```python
from build123d import *

# Parameters (mm, degrees)
CUT_EXTRUDE1_DEPTH = 3
CHAMFER1_SIZE      = 0.5


with BuildPart() as part:
    # Sketch1 → Revolve1 (revolve)
    with BuildSketch(Plane.XY):
        Polygon((0, 0), (0, 6.55), (12, 6.55), (12, 9.5), (17, 9.5), (17, 0), align=None)
    revolve(axis=Axis((17, 0, 0), (-1, 0, 0)))

    # Sketch2 → Cut-Extrude1 (cut)
    with BuildSketch(Plane(origin=(17, 0, 0), x_dir=(0, 0, -1), z_dir=(1, 0, 0))):
        Polygon((0, 4.041451884), (-3.5, 2.020725942), (-3.5, -2.020725942), (0, -4.041451884), (3.5, -2.020725942), (3.5, 2.020725942), align=None)
    extrude(amount=-CUT_EXTRUDE1_DEPTH, mode=Mode.SUBTRACT)

    # Chamfer1
    chamfer1_edges = [part.edges().sort_by_distance(p)[0] for p in [
        (17, -9.5, 0),
        (12, -9.5, 0),
        (0, -6.55, 0),
    ]]
    chamfer(chamfer1_edges, length=CHAMFER1_SIZE)


solid = part.part
```
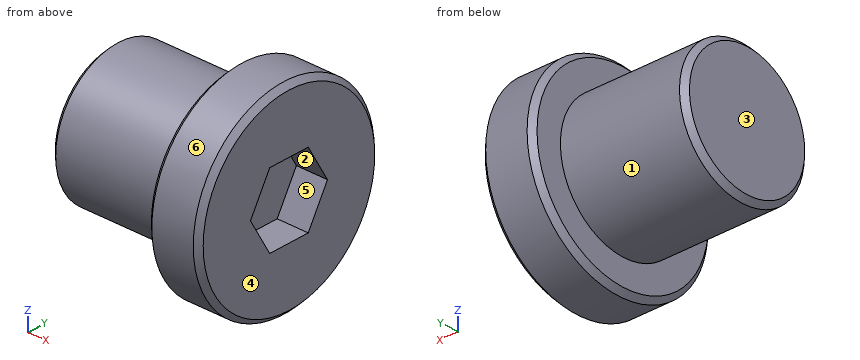
The listing builds one solid part. Answer for the finished solid, in the listing's coordinates (mm). Face numbers are marked on the shaded views. A direction names the side the tool comes from. Round coordinates to 2 decimals unless told otherwise and drop trailing zeros. Order: outer loops, then holes, each group sorted by start corner. A loop starts at its lowest first (then second) coordinate and runs counter-clockwise, first axis right, second up. Notation, with made-up numbers: (89.25, 29) -> (113.25, 29) arc R28 cw to (113.25, 59) -> close; hole circle Ø3 at (49, 73). An arc over 180 degrees is marked (long way). Answer as CSV lines item,"result".
Q1. Consider line 1 (X direction, y = -3.75, z = -4.75); line 2 (X direction, y = 8.5, z = 1.25); line 3 (Y direction, x = 9, z = 0). Determine where each line is inside the solid, lowest interval first. Write a range as from..to.
Computed values:
line 1,"x = 0..17"
line 2,"x = 12..17"
line 3,"y = -6.55..6.55"
Q2. For a pull along Y with two mould halves and no side action, classify the marked faces 4, 5 and 6 as +Y half, -Y half, draft (parallel to the pull), parting line (faces both ways), or undercut.
Computed values:
face 4,"draft"
face 5,"undercut"
face 6,"parting line"
Q3. A cutting plane is placed at A-A on y = 0. Determine the outline of the cut face in (x, z).
Computed values:
outline,"(0, -6.05) -> (0.5, -6.55) -> (12, -6.55) -> (12, -9) -> (12.5, -9.5) -> (16.5, -9.5) -> (17, -9) -> (17, -3.5) -> (14, -3.5) -> (14, 3.5) -> (17, 3.5) -> (17, 9) -> (16.5, 9.5) -> (12.5, 9.5) -> (12, 9) -> (12, 6.55) -> (0.5, 6.55) -> (0, 6.05) -> close"
Q4. A cutting plane is placed at B-B on x = 5. Determine the outline of the cut face in (y, z), plus the area to 3 significant figures.
Computed values:
outline,"circle Ø13.1 at (0, 0)"
area,"135 mm^2"
Q5. Given pin 1 (10 mm diameter, centred on x = 12, y = -1.5, fed in from +Z); pin 2 (3.5 mm diameter, centred on y = 0.5, z = -1, fed in from +X); pin 3 (6 mm diameter, centred on x = 2, z = -3.5, fed in from +Y); pin 4 (1 mm diameter, centred on x = 12.5, z = 5.5, fed in from -Y), each flat-ended and moving along its own axis, determine where each tip first touches the part or whether it passes through.
Computed values:
pin 1,"stops at z = 9.5"
pin 2,"stops at x = 14"
pin 3,"stops at y = 6.53"
pin 4,"stops at y = -8.08"
Q6. Which of the six approach directions +Z, -Z, +X, -X, +Y, -Y give full straight-line access (tool end or side, diameter ignored) to the marked faces 1, 2 and 3?
Computed values:
face 1,"-X"
face 2,"+X"
face 3,"+Z, -Z, -X, +Y, -Y"
